```python
from build123d import *

# Parameters (mm, degrees)
SKETCH1_R           = 12.5
BOSS_EXTRUDE1_DEPTH = 20
CHAMFER1_SIZE       = 1


with BuildPart() as part:
    # Sketch1 → Boss-Extrude1 (new body)
    with BuildSketch(Plane.XY):
        Circle(SKETCH1_R)
        with BuildLine():
            Line((-2, 7.5), (2, 7.5))
            ThreePointArc((2, 7.5), (9.5, 0), (2, -7.5))
            Line((2, -7.5), (-2, -7.5))
            ThreePointArc((-2, -7.5), (-9.5, 0), (-2, 7.5))
        make_face(mode=Mode.SUBTRACT)
    extrude(amount=BOSS_EXTRUDE1_DEPTH)

    # Chamfer1
    chamfer1_edges = [part.edges().sort_by_distance(p)[0] for p in [
        (0, 7.5, 20),
        (-9.5, 0, 20),
        (0, -7.5, 20),
        (9.5, 0, 20),
    ]]
    chamfer(chamfer1_edges, length=CHAMFER1_SIZE)


solid = part.part
```
The model under review builds one solid part; all positions refer to its coordinate system, in mm. A direction names the side the tool comes from. Coordinates: 2 decimals unless noted, no trailing zeros. Write each loop counter-clockwise with the first axis right and the second up, starting at its lowest first coordinate (ties: lowest second). Pieces come first, ordered by that corner, then holes.
1) We need section D-D on x = -11. State the section outline as (y, z) points, then the cut area to 3 significant figures.
2) We need section B-B on x = 0. State the section outline as (y, z) points.
3) Clearance check with flat-ended pins moving along their axes: pin 1 Ø4 at (x, z) = (-4.5, 8) entering from -Y; pin 2 Ø1 at (y, z) = (-4.5, 15.5) entering from +X; pin 3 Ø12 at (y, z) = (-8.5, 9) entering from -X. State where each tip first meets the part, or that it passes through.
4) We need section A-A on y = 0. State the section outline as (x, z) points, then the cut area to 3 significant figures.
5) Machinability: for faces 1 (the face through (-9.5, -0.16, 9.37)), 2 (the face through (0, -8, 0)), 3 (the face through (9.7, 0.2, 19.2)), which of the approach directions +Z, -Z, +X, -X, +Y, -Y give a long, thin tool a straight path to every point of the face, cutting with its end or side? Answer none if there is none.
6) We need section C-C on z = 16.75. State the section outline as (x, y) points, then the cut area to 3 significant figures.
7) The part is to be moulded in two halves that separate along Y. For faces 4 (the face through (11.923, 3.755, 9.86)), 5 (the face through (2, 9, 20)), 6 (the face through (0, -8, 19.5)), say which applies: pulls with the +Y half, pulls with the -Y half, needs draft (parallel to the pull), parting line crosses it, or undercut.
8) To check wall thickness, follow probe 1 along Y at (x, z) = (0, 4.25); probe 2 along Y at (x, z) = (-2.5, 11.25); probe 3 along X at (y, z) = (3, 3.25). State the ranges of each line that lie inside material, in increasing order.
Answer list:
1. outline: (-5.94, 0) - (5.94, 0) - (5.94, 20) - (-5.94, 20) - close
1. area: 237 mm2
2. outline: (-12.5, 0) - (-7.5, 0) - (-7.5, 19) - (-8.5, 20) - (-12.5, 20) - close; (7.5, 0) - (12.5, 0) - (12.5, 20) - (8.5, 20) - (7.5, 19) - close
3. pin 1: stops at y = -12.25
3. pin 2: stops at x = 11.84
3. pin 3: stops at x = -12.25
4. outline: (-12.5, 0) - (-9.5, 0) - (-9.5, 19) - (-10.5, 20) - (-12.5, 20) - close; (9.5, 0) - (12.5, 0) - (12.5, 20) - (10.5, 20) - (9.5, 19) - close
4. area: 119 mm2
5. face 1: +Z, -Z
5. face 2: -Z, +X, -X, +Y, -Y
5. face 3: +Z
6. outline: circle Ø25 at (0, 0); hole (-2, -7.5) - (2, -7.5) arc R7.5 ccw to (2, 7.5) - (-2, 7.5) arc R7.5 ccw to start
6. area: 254 mm2
7. face 4: parting line crosses it
7. face 5: needs draft
7. face 6: undercut
8. probe 1: y = -12.5 to -7.5, 7.5 to 12.5
8. probe 2: y = -12.25 to -7.48, 7.48 to 12.25
8. probe 3: x = -12.13 to -8.87, 8.87 to 12.13
